Source: CAD feature listing. Evaluate the final solid. Frame: model axes, mm. Face numbers are marked on the shaded views. A direction names the side the tool comes from. Round coordinates to 2 decimals unless told otherwise and drop trailing zeros. Order: outer loops, then holes, each group sorted by start corner. A loop starts at its lowest first (then second) coordinate and runs counter-clockwise, first axis right, second up. Notation, with made-up numbers: (65.5, 56.25) - (109.5, 56.25) arc R25 cw to (109.5, 91.25) - close; hole circle Ø7 at (24.5, 42). An arc over 180 degrees is marked (long way). Use one line per item in the form item = value. Start each with the question number.
Q1. Cut plane A-A, the plane x = 21. Return the cut outline in (y, z).
Q2. Draft query along Y for the marked faces 1, 2 and 3. Return one class per face: released by +Y, released by -Y, zero draft, split by the parting line, or undercut.
Q3. Cut plane C-C, the plane y = 30. Return the cut outline in (x, z).
Q4. Cut plane B-B, the plane x = 66.5. Return the cut outline in (y, z).
Q5. Pin query (flat end, axial travel): pin 1 Ø8 at (x, z) = (64, 50.5) entering from -Y; pin 2 Ø18 at (y, z) = (28.5, 47) entering from -X; pin 3 Ø9 at (x, y) = (18, 26) entering from +Z; pin 4 Ø6 at (y, z) = (33.5, 45) entering from -X. Return the tip coordinate at first contact, or that it passes through.
Q6. Set-up query: the marked faces 4, 5 and 6. Return all of +Z, -Z, +X, -X, +Y, -Y with unobstructed straight access to the full face (end or side cutting, diameter ignored); none if empty.
Q7. Cut plane D-D, the plane z = 18. Return the cut outline in (x, y), and give its area (3 significant figures).
Q8. Ray query, line 1 (Y direction, x = 63.3, z = 45); line 2 (Y direction, x = 66.5, z = 45); line 3 (Z direction, x = 40.5, y = 21). Return the intervals inside material, ascending. Write a range as [from, to].
from build123d import *

# Parameters (mm, degrees)
BASE_PLATE_SKETCH_W = 80
BASE_PLATE_SKETCH_H = 60
BASE_PLATE_DEPTH    = 15
UPRIGHT_BLOCK_DEPTH = 20
RECESS_30_SKETCH_R  = 15
RECESS_30_DEPTH     = 5
RECESS_20_SKETCH_R  = 10
RECESS_20_DEPTH     = 5
SLOT_30_DEPTH       = 5
SLOT_STEP_20_DEPTH  = 10
SIDE_BOSS_DEPTH     = 10
ROUNDED_BOSS_DEPTH  = 10


with BuildPart() as part:
    # Base Plate Sketch → Base Plate (new body)
    with BuildSketch(Plane.XY):
        with Locations((40, 30)):
            Rectangle(BASE_PLATE_SKETCH_W, BASE_PLATE_SKETCH_H)
    extrude(amount=BASE_PLATE_DEPTH)

    # Upright Block Sketch → Upright Block (add)
    with BuildSketch(Plane(origin=(80, 0, 0), x_dir=(0, 0, -1), z_dir=(1, 0, 0))):
        with BuildLine():
            Line((-15, 60), (-45, 60))
            ThreePointArc((-45, 60), (-75, 30), (-45, 0))
            Line((-45, 0), (-15, 0))
            Line((-15, 0), (-15, 60))
        make_face()
    extrude(amount=-UPRIGHT_BLOCK_DEPTH)

    # Recess Ø30 Sketch → Recess Ø30 (cut)
    with BuildSketch(Plane.ZY.offset(-60)):
        with Locations((45, 30)):
            Circle(RECESS_30_SKETCH_R)
    extrude(amount=-RECESS_30_DEPTH, mode=Mode.SUBTRACT)

    # Recess Ø20 Sketch → Recess Ø20 (cut)
    with BuildSketch(Plane.ZY.offset(-65)):
        with Locations((45, 30)):
            Circle(RECESS_20_SKETCH_R)
    extrude(amount=-RECESS_20_DEPTH, mode=Mode.SUBTRACT)

    # Slot 30 Sketch → Slot 30 (cut)
    with BuildSketch(Plane.XY.offset(15)):
        with BuildLine():
            Line((0, 45), (0, 15))
            Line((0, 15), (30, 15))
            ThreePointArc((30, 15), (45, 30), (30, 45))
            Line((30, 45), (0, 45))
        make_face()
    extrude(amount=-SLOT_30_DEPTH, mode=Mode.SUBTRACT)

    # Slot Step 20 Sketch → Slot Step 20 (cut)
    with BuildSketch(Plane.XY.offset(10)):
        with BuildLine():
            Line((0, 40), (30, 40))
            ThreePointArc((30, 40), (40, 30), (30, 20))
            Line((30, 20), (0, 20))
            Line((0, 20), (0, 40))
        make_face()
    extrude(amount=-SLOT_STEP_20_DEPTH, mode=Mode.SUBTRACT)

    # Side Boss Sketch → Side Boss (add)
    with BuildSketch(Plane.XZ):
        Polygon((60, 45), (40, 15), (60, 15), align=None)
    extrude(amount=-SIDE_BOSS_DEPTH)

    # Rounded Boss Sketch → Rounded Boss (add)
    with BuildSketch(Plane(origin=(0, 60, 0), x_dir=(1, 0, 0), z_dir=(0, 1, 0))):
        Polygon((40, -15), (60, -15), (60, -45), align=None)
    extrude(amount=-ROUNDED_BOSS_DEPTH)


solid = part.part
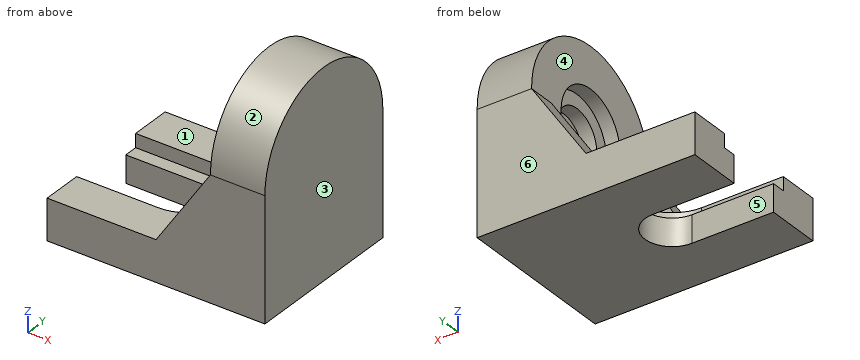
Completed:
q1.outline = (0, 0) - (20, 0) - (20, 10) - (15, 10) - (15, 15) - (0, 15) - close; (40, 0) - (60, 0) - (60, 15) - (45, 15) - (45, 10) - (40, 10) - close
q2.face_1 = undercut
q2.face_2 = split by the parting line
q2.face_3 = zero draft
q3.outline = (40, 0) - (80, 0) - (80, 75) - (60, 75) - (60, 60) - (65, 60) - (65, 55) - (70, 55) - (70, 35) - (65, 35) - (65, 30) - (60, 30) - (60, 15) - (45, 15) - (45, 10) - (40, 10) - close
q4.outline = (0, 0) - (60, 0) - (60, 45) arc R30 ccw to (0, 45) - close; hole circle Ø20 at (30, 45)
q5.pin_1 = 0.04
q5.pin_2 = 65
q5.pin_3 = through
q5.pin_4 = 70
q6.face_4 = +Z, -X
q6.face_5 = +Z, -Z, -X
q6.face_6 = +Z, -Z, +X, -X, +Y
q7.outline = (42, 0) - (80, 0) - (80, 60) - (42, 60) - (42, 50) - (60, 50) - (60, 10) - (42, 10) - close
q7.area = 1,560 mm2
q8.line_1 = [0, 15], [45, 60]
q8.line_2 = [0, 20], [40, 60]
q8.line_3 = [0, 10]
